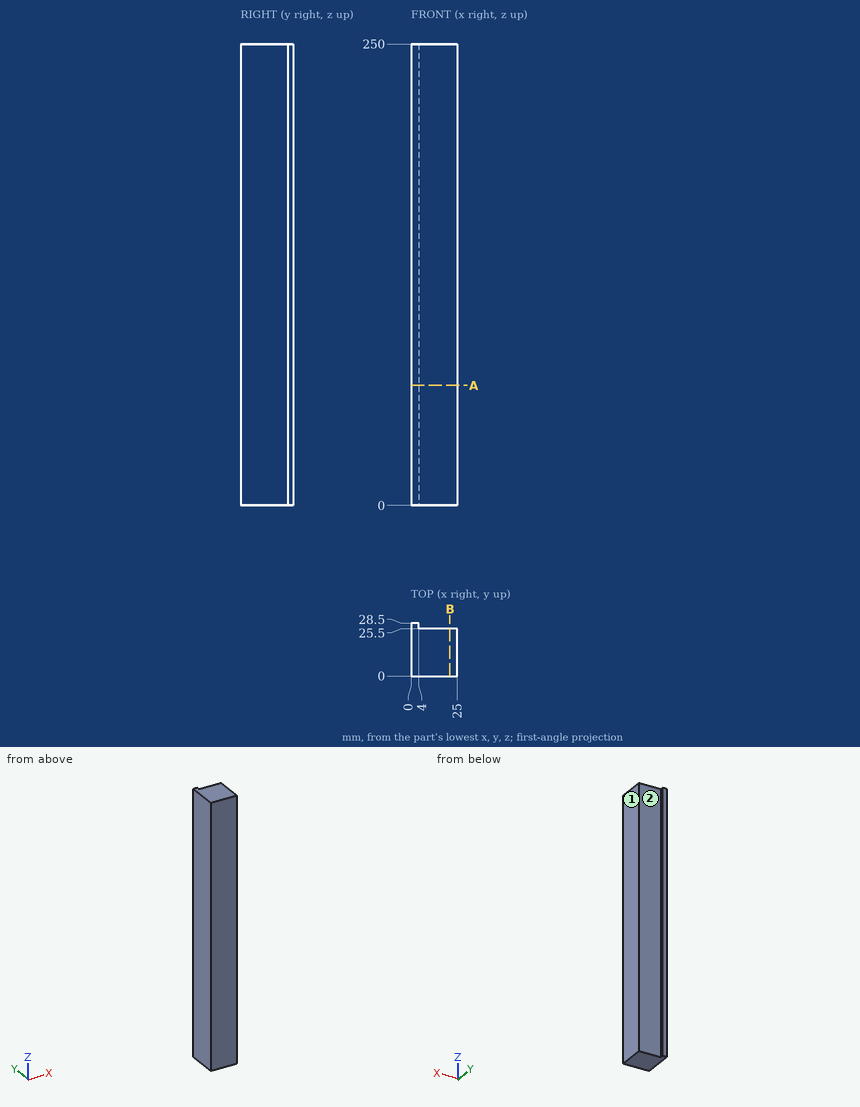
Answer from the drawing. Dimensions are ordinates in mm from the lowest x, y and z of the part. A direction names the side the tool comes from. Coordinates: 2 decimals unless noted, no trailing zeros. Loops run counter-clockwise (first coordinate to the right, second up) from the corner with the lowest first, then second, coordinate; pieces in that order, holes last. Notation, with made-up numbers: (86.5, 13.5) - (117.5, 13.5) arc R16 ccw to (117.5, 25.5) - close; hole circle Ø2 at (44, 62). An arc over 180 degrees is marked (long way). Answer in a Markdown table with one row per item.
1. Given pin 1 (0.9 mm diameter, centred on y = 27, z = 173.5, fed in from +X); pin 2 (1 mm diameter, centred on x = 11, z = 45.5, fed in from +Y), each flat-ended and moving along its own axis, determine where each tip first touches the part or whether it passes through.
Conclusion:
| item | result |
|---|---|
| pin 1 | stops at x = 4 |
| pin 2 | stops at y = 25.5 |
2. Straight lines are drawn through the part: line 1 (Y direction, x = 13.75, z = 150); line 2 (X direction, y = 27.5, z = 234.5). For each, find the intervals that lie inside material, in ascending order.
Conclusion:
| item | result |
|---|---|
| line 1 | y = 0 to 25.5 |
| line 2 | x = 0 to 4 |
3. Find section B-B, the plane x = 21. Write down the section's boundary in (y, z), then the cut area to 4 significant figures.
Conclusion:
| item | result |
|---|---|
| outline | (0, 0) - (25.5, 0) - (25.5, 250) - (0, 250) - close |
| area | 6,375 mm² |
4. Which of the six approach directions +Z, -Z, +X, -X, +Y, -Y give full straight-line access (tool end or side, diameter ignored) to the marked faces 1 and 2?
Conclusion:
| item | result |
|---|---|
| face 1 | +Z, -Z, +X, +Y, -Y |
| face 2 | +Z, -Z, +X, +Y |
5. Find section A-A, the plane z = 65. Write down the section's boundary in (x, y), then the cut area to 4 significant figures.
Conclusion:
| item | result |
|---|---|
| outline | (0, 0) - (25, 0) - (25, 25.5) - (4, 25.5) - (4, 28.5) - (0, 28.5) - close |
| area | 649.5 mm² |
